Study the drawing (mm; zero at the part's minimum x, y, z) and answer. Give positions to 0.01 mm unless a question says otherwise; leave off trailing zeros. Write each loop counter-clockwise with the first axis right and the second up, starting at its lowest first coordinate (ties: lowest second). Pieces come first, ordered by that corner, then holes. Notation, with made-up numbers: M 16.25,84.25 L 40.25,84.25 A13 ccw 40.25,92.25 Z; hole C 10,-21 d2. An arc over 180 degrees is marked long. Use a Markdown table: item, result. Add a question column.
Item 1: A cutting plane is placed at B-B on z = 3.75. Determine the outline of the cut face in (x, y), then the cut area to 3 significant figures.
Item 2: A cutting plane is placed at A-A on y = 27. Determine the outline of the cut face in (x, z).
Item 3: A cutting plane is placed at C-C on x = 51. Determine the outline of the cut face in (y, z), then the cut area to 3 significant figures.
Item 4: Consider probe 1 along X at (y, z) = (28.75, 9.5); probe 2 along Y at (x, z) = (93.5, 12.25); probe 3 along Y at (x, z) = (15.5, 4.5). Determine where each line is inside the solid, lowest interval first. Write a range as [from, to].
Item 5: Given P1, Ø3, axis at x = 94.5, z = 9, coming from the -Y side; P2, Ø5, axis at x = 88.5, z = 9.5, coming from the -Y side; P3, Ø5, axis at y = 18.5, z = 14.5, coming from the -X side, each flat-ended and moving along its own axis, determine where each tip first touches the part or whether it passes through.
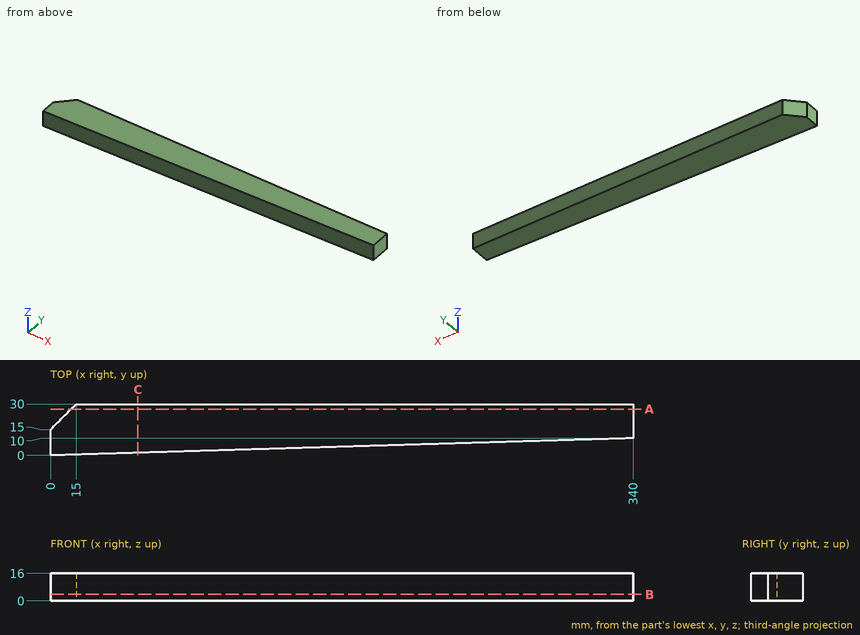
Filled in:
| question | item | result |
|---|---|---|
| 1 | outline | M 0,0 L 340,10 L 340,30 L 15,30 L 0,15 Z |
| 1 | area | 8,390 mm² |
| 2 | outline | M 12,0 L 340,0 L 340,16 L 12,16 Z |
| 3 | outline | M 1.5,0 L 30,0 L 30,16 L 1.5,16 Z |
| 3 | area | 456 mm² |
| 4 | probe 1 | [13.75, 340] |
| 4 | probe 2 | [2.75, 30] |
| 4 | probe 3 | [0.46, 30] |
| 5 | P1 | y = 2.74 |
| 5 | P2 | y = 2.53 |
| 5 | P3 | x = 1 |
